CAD build for the part. Positions are in the model's coordinates, mm. Face numbers are marked on the shaded views. Round coordinates to 2 decimals unless told otherwise and drop trailing zeros. Order: outer loops, then holes, each group sorted by start corner. A loop starts at its lowest first (then second) coordinate and runs counter-clockwise, first axis right, second up. Notation, with made-up numbers: (-4, 32) - (23, 32) arc R30 ccw to (23, 64) - close; hole circle Ø2 at (-38, -26). An arc over 180 degrees is marked (long way). Write item = value, one per line.
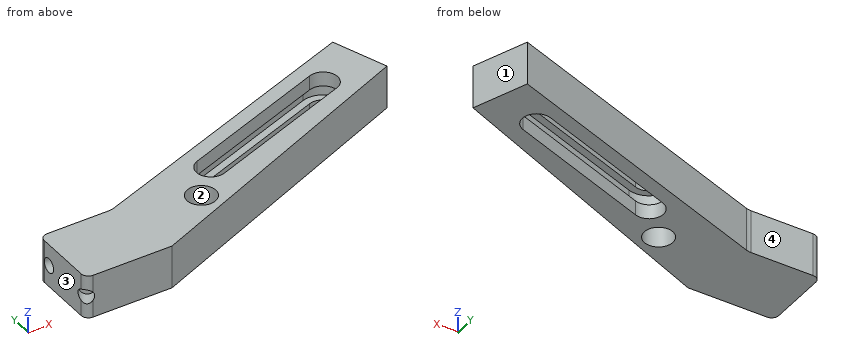
from build123d import *

# Parameters (mm, degrees)
BOSS_EXTRUDE1_DEPTH = 15
FILLET1_R           = 10
FILLET2_R           = 5
SKETCH2_R           = 5
CUT_EXTRUDE1_DEPTH  = 10
SKETCH3_R           = 5
CUT_EXTRUDE2_DEPTH  = 10
SKETCH5_R           = 10
BOSS_EXTRUDE3_DEPTH = 10
SKETCH6_R           = 7.5
BOSS_EXTRUDE4_DEPTH = 5
SKETCH7_R           = 10
BOSS_EXTRUDE5_DEPTH = 2
SKETCH8_R           = 10
CUT_EXTRUDE3_DEPTH  = 80
CUT_EXTRUDE4_DEPTH  = 5
SKETCH10_W          = 33.070840011
SKETCH10_H          = 51.47652372
CUT_EXTRUDE5_DEPTH  = 50


with BuildPart() as part:
    # Sketch1 → Boss-Extrude1 (new, symmetric)
    with BuildSketch(Plane.XY):
        Polygon((0, 0), (0, 50), (50, 50), (250.63503339, 123.025180105), (264.315839123, 85.437475274), (60, 0), align=None)
        with BuildLine():
            Line((118.808982902, 64.402643902), (220.866512245, 101.548546765))
            ThreePointArc((220.866512245, 101.548546765), (233.683639886, 95.571821991), (227.706915111, 82.75469435))
            Line((227.706915111, 82.75469435), (125.649385769, 45.608791486))
            ThreePointArc((125.649385769, 45.608791486), (112.832258128, 51.585516261), (118.808982902, 64.402643902))
        make_face(mode=Mode.SUBTRACT)
    extrude(amount=BOSS_EXTRUDE1_DEPTH, both=True)

    # Fillet1
    fillet1_edges = [part.edges().sort_by_distance(p)[0] for p in [
        (50, 50, 0),
    ]]
    fillet(fillet1_edges, radius=FILLET1_R)

    # Fillet2
    fillet2_edges = [part.edges().sort_by_distance(p)[0] for p in [
        (0, 0, 0),
        (0, 50, 0),
    ]]
    fillet(fillet2_edges, radius=FILLET2_R)

    # Sketch2 → Cut-Extrude1 (cut)
    with BuildSketch(Plane(origin=(1.166172543, 1.605098805, 0), x_dir=(0, 0, -1), z_dir=(-0.587785252292477, -0.8090169943749446, 0))):
        with Locations(Location((0, 0, 0), (0, 0, 90))):
            Circle(SKETCH2_R)
    extrude(amount=-CUT_EXTRUDE1_DEPTH, mode=Mode.SUBTRACT)

    # Sketch3 → Cut-Extrude2 (cut)
    with BuildSketch(Plane.ZY):
        with Locations((0, 40)):
            Circle(SKETCH3_R)
    extrude(amount=-CUT_EXTRUDE2_DEPTH, mode=Mode.SUBTRACT)

    # Sketch5 → Boss-Extrude3 (add)
    with BuildSketch(Plane(origin=(0, 0, -15), x_dir=(-1, 0, 0), z_dir=(0, 0, -1))):
        with Locations((-15, 25.111581997)):
            Circle(SKETCH5_R)
    extrude(amount=BOSS_EXTRUDE3_DEPTH)

    # Sketch6 → Boss-Extrude4 (add)
    with BuildSketch(Plane(origin=(0, 0, -25), x_dir=(-1, 0, 0), z_dir=(0, 0, -1))):
        with Locations((-15, 25.111581997)):
            Circle(SKETCH6_R)
    extrude(amount=BOSS_EXTRUDE4_DEPTH)

    # Sketch7 → Boss-Extrude5 (add)
    with BuildSketch(Plane(origin=(0, 0, -30), x_dir=(-1, 0, 0), z_dir=(0, 0, -1))):
        with Locations((-15, 25.111581997)):
            Circle(SKETCH7_R)
    extrude(amount=BOSS_EXTRUDE5_DEPTH)

    # Sketch8 → Cut-Extrude3 (cut)
    with BuildSketch(Plane.XY.offset(15)):
        with Locations((102.166886521, 33.891313111)):
            Circle(SKETCH8_R)
    extrude(amount=-CUT_EXTRUDE3_DEPTH, mode=Mode.SUBTRACT)

    # Sketch9 → Cut-Extrude4 (cut, symmetric)
    with BuildSketch(Plane.XY):
        with BuildLine():
            Line((127.359486485, 40.910328382), (229.417015828, 78.056231246))
            ThreePointArc((229.417015828, 78.056231246), (238.38210299, 97.281922707), (219.156411528, 106.247009869))
            Line((219.156411528, 106.247009869), (117.098882186, 69.101107006))
            ThreePointArc((117.098882186, 69.101107006), (108.133795024, 49.875415544), (127.359486485, 40.910328382))
        make_face()
        with BuildLine():
            Line((220.866512245, 101.548546765), (118.808982902, 64.402643902))
            ThreePointArc((118.808982902, 64.402643902), (112.832258128, 51.585516261), (125.649385769, 45.608791486))
            Line((125.649385769, 45.608791486), (227.706915111, 82.75469435))
            ThreePointArc((227.706915111, 82.75469435), (233.683639886, 95.571821991), (220.866512245, 101.548546765))
        make_face(mode=Mode.SUBTRACT)
    extrude(amount=CUT_EXTRUDE4_DEPTH, both=True, mode=Mode.SUBTRACT)

    # Sketch10 → Cut-Extrude5 (cut)
    with BuildSketch(Plane.ZY):
        with Locations((-31.535420006, 25.73826186)):
            Rectangle(SKETCH10_W, SKETCH10_H)
    extrude(amount=-CUT_EXTRUDE5_DEPTH, mode=Mode.SUBTRACT)


solid = part.part
(1) Drop flat-ended pins along their axis: pin 1 (12 mm diameter, centred on y = 53, z = 1.5, fed in from +X); pin 2 (6 mm diameter, centred on x = 233, z = -0.5, fed in from -Y); pin 3 (9 mm diameter, centred on x = 29, z = -1, fed in from +Y). Give the stop position or say it passes through.
Solved:
pin_1 = 201.09
pin_2 = 71.09
pin_3 = 50
(2) Probe line 1 along Z through (x, y) = (5, 40); line 2 along Y through (x, z) = (15, -4.5); line 3 along Y through (x, z) = (213.5, -0.5). List the from-to ranges inside material, lowest first.
Solved:
line_1 = -15 to -5, 5 to 15
line_2 = 0 to 50
line_3 = 64.19 to 72.26, 104.19 to 109.51
(3) Band-saw the part on A-A on x = 225. List the corners of the cut face in (y, z).
Solved:
outline = (69, -15) - (81.77, -15) - (81.77, -5) - (76.45, -5) - (76.45, 5) - (81.77, 5) - (81.77, 15) - (69, 15) - close; (102.13, -15) - (113.69, -15) - (113.69, 15) - (102.13, 15) - (102.13, 5) - (107.13, 5) - (107.13, -5) - (102.13, -5) - close
(4) Band-saw the part on B-B on y = 60.5. List the corners of the cut face in (x, z).
Solved:
outline = (78.85, -15) - (113.87, -15) - (113.87, -5) - (108.27, -5) - (108.27, 5) - (113.87, 5) - (113.87, 15) - (78.85, 15) - close; (166.56, -15) - (204.68, -15) - (204.68, 15) - (166.56, 15) - (166.56, 5) - (181.18, 5) - (181.18, -5) - (166.56, -5) - close
(5) Band-saw the part on C-C on z = 12. List the corners of the cut face in (x, y).
Solved:
outline = (0, 5) arc R5 ccw to (5, 0) - (60, 0) - (264.32, 85.44) - (250.64, 123.03) - (51.66, 50.6) arc R10 cw to (48.24, 50) - (5, 50) arc R5 ccw to (0, 45) - close; hole circle Ø20 at (102.17, 33.89); hole (118.81, 64.4) arc R10 ccw to (125.65, 45.61) - (227.71, 82.75) arc R10 ccw to (220.87, 101.55) - close
(6) Pull direction X, two halves, no side cores. Call the marked faces 1, 2, 3 and 4: released by +X, released by -X, zero draft, split by the parting line, or undercut.
Solved:
face_1 = released by +X
face_2 = undercut
face_3 = released by -X
face_4 = zero draft
(7) Band-saw the part on D-D on x = 103. List the corners of the cut face in (y, z).
Solved:
outline = (17.98, -15) - (23.93, -15) - (23.93, 15) - (17.98, 15) - close; (43.86, -15) - (69.29, -15) - (69.29, 15) - (43.86, 15) - close
